Design review of the part shown in the three views and the two pictorial views. Dimensions are in mm from the part's minimum x, y and z. A direction names the side the tool comes from. Round coordinates to 2 decimals unless told otherwise and drop trailing zeros. Loops run counter-clockwise (first coordinate to the right, second up) from the corner with the lowest first, then second, coordinate; pieces in that order, holes last. Notation, with made-up numbers: (18, -12.5) -> (63, -12.5) arc R11 cw to (63, 0.5) -> close; hole circle Ø7 at (89.5, 43.5). An arc over 180 degrees is marked (long way). Use CSV: the item, a comma, the result in double quotes. Start each with the question number.
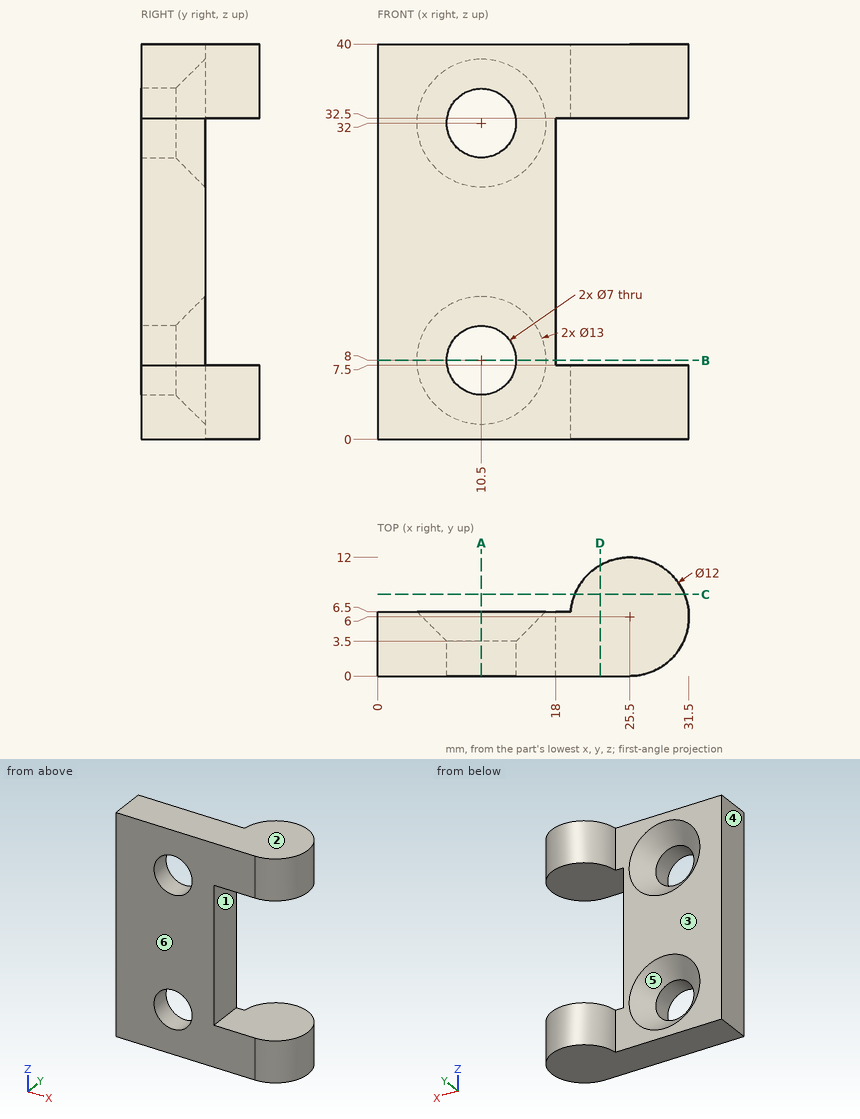
1. Take a section at B-B, the plane z = 8. Give the boundary of the cut face in (x, y).
2. Take a section at C-C, the plane y = 8.25. Give the boundary of the cut face in (x, z).
3. For the marked faces 1, 2 and 3, list the 3-axis set-ups (+Z, -Z, +X, -X, +Y, -Y) from which the entire face can be reached by the end or side of a thin tool; tool diameter is ignored.
4. For line 1 along Z through (x, y) = (23.5, 2.75); line 2 along X through (y, z) = (0.7, 8); line 3 along Z through (x, y) = (11.5, 4.25), list the stretches that pass through material, from the lowest coordinate up. Write a range as from..to.
5. The part is to be moulded in two halves that separate along X. For the marked faces 4, 5 and 6, say which applies: pulls with the +X half, pulls with the -X half, needs draft (parallel to the pull), parting line crosses it, or undercut.
6. Clearance check with flat-ended pins moving along their axes: P1, Ø7, axis at y = 2, z = 17.5, coming from the +X side; P2, Ø11, axis at x = 10.5, z = 8, coming from the +Y side; P3, Ø6, axis at x = 23, y = 5, coming from the -Z side; P4, Ø15.5, axis at x = 9, z = 13.5, coming from the +Y side. State where each tip first meets the part, or that it passes through.
7. Take a section at D-D, the plane x = 22.5. Give the boundary of the cut face in (y, z), then the cut area to 3 significant figures.
8. Take a section at A-A, the plane x = 10.5. Give the boundary of the cut face in (y, z), then the cut area to 3 significant figures.
Results:
1,outline,"(0, 0) -> (7, 0) -> (7, 3.5) -> (4, 6.5) -> (0, 6.5) -> close; (14, 0) -> (18, 0) -> (18, 6.5) -> (17, 6.5) -> (14, 3.5) -> close"
2,outline,"(19.94, 0) -> (31.06, 0) -> (31.06, 7.5) -> (19.94, 7.5) -> close; (19.94, 32.5) -> (31.06, 32.5) -> (31.06, 40) -> (19.94, 40) -> close"
3,face 1,"+X, +Y, -Y"
3,face 2,"+Z, +X, -X, +Y, -Y"
3,face 3,"+Z, -Z, -X, +Y"
4,line 1,"0..7.5, 32.5..40"
4,line 2,"0..7, 14..18"
4,line 3,"0..3.87, 12.13..27.87, 36.13..40"
5,face 4,"pulls with the -X half"
5,face 5,"undercut"
5,face 6,"needs draft"
6,P1,"x = 18"
6,P2,"y = 5.5"
6,P3,"z = 0"
6,P4,"y = 6.5"
7,outline,"(0, 0) -> (11.2, 0) -> (11.2, 7.5) -> (0, 7.5) -> close; (0, 32.5) -> (11.2, 32.5) -> (11.2, 40) -> (0, 40) -> close"
7,area,"168 mm²"
8,outline,"(0, 0) -> (6.5, 0) -> (6.5, 1.5) -> (3.5, 4.5) -> (0, 4.5) -> close; (0, 11.5) -> (3.5, 11.5) -> (6.5, 14.5) -> (6.5, 25.5) -> (3.5, 28.5) -> (0, 28.5) -> close; (0, 35.5) -> (3.5, 35.5) -> (6.5, 38.5) -> (6.5, 40) -> (0, 40) -> close"
8,area,"151 mm²"
